```python
from build123d import *

# Parameters (mm, degrees)
SHAFT_SECTION_A_PROFILE_10_R = 5
SHAFT_SECTION_A_10X64_DEPTH  = 64
COLLAR_PROFILE_24_R          = 12
COLLAR_24X2_DEPTH            = 2
SHAFT_START                  = 80
SHAFT_SECTION_B_PROFILE_10_R = 5
SHAFT_SECTION_B_10X80_DEPTH  = 80
HEAD_PROFILE_18_R            = 9
HEAD_18X4_DEPTH              = 4


with BuildPart() as part:
    # Shaft Section A Profile Ø10 → Shaft Section A Ø10x64 (new body)
    with BuildSketch(Plane(origin=(0, 0, 0), x_dir=(0, 0, -1), z_dir=(1, 0, 0))):
        Circle(SHAFT_SECTION_A_PROFILE_10_R)
    extrude(amount=SHAFT_SECTION_A_10X64_DEPTH)

    # Collar Profile Ø24 → Collar Ø24x2 (add)
    with BuildSketch(Plane.ZY):
        Circle(COLLAR_PROFILE_24_R)
    extrude(amount=COLLAR_24X2_DEPTH)

    # Shaft Section B Profile Ø10 → Shaft Section B Ø10x80 (add)
    with BuildSketch(Plane.ZY.offset(2).offset(SHAFT_START)):
        with Locations(Location((0, 0, 0), (0, 0, 180))):
            Circle(SHAFT_SECTION_B_PROFILE_10_R)
    extrude(amount=-SHAFT_SECTION_B_10X80_DEPTH)

    # Head Profile Ø18 → Head Ø18x4 (add)
    with BuildSketch(Plane.ZY.offset(82)):
        Circle(HEAD_PROFILE_18_R)
    extrude(amount=HEAD_18X4_DEPTH)


solid = part.part
```
Geometry check sheet. Reference: the model listing, model coordinates, mm. A direction names the side the tool comes from. Round coordinates to 2 decimals unless told otherwise and drop trailing zeros. Order: outer loops, then holes, each group sorted by start corner. A loop starts at its lowest first (then second) coordinate and runs counter-clockwise, first axis right, second up. Notation, with made-up numbers: (37.5, 31) - (83.5, 31) arc R27 cw to (83.5, 52) - close; hole circle Ø8 at (45.25, 23.25). An arc over 180 degrees is marked (long way). Use a Markdown table: item, result. Add a question column.
(1) Sectioned sample at A-A, the plane y = 7.5. Enter the section's corners in (x, z), and give its area (3 significant figures).
(2) Tool access check on faces 1 (the flat face through (64, 0, 0)), 2 (the flat face through (-86, 0, 0)), 3 (the cylindrical face through (-83.972, 8.923, -1.172)), 4 (the flat face through (-2, 0.2, 5.2)), 5 (the flat face through (0, 0.2, 5.2)). Record the directions out of +Z, -Z, +X, -X, +Y, -Y that give a thin tool (end or side, any length) a straight path to the whole face; none if there is none.
(3) Depth check by flat-ended pin: pin 1 (2 mm diameter, centred on x = 42.5, z = -5.5, fed in from -Y); pin 2 (4 mm diameter, centred on x = 39, y = 8.5, fed in from -Z); pin 3 (4 mm diameter, centred on x = 17.5, z = 6.5, fed in from +Y); pin 4 (5 mm diameter, centred on x = 48, y = -5, fed in from +Z). Enter the tip coordinate at first touch or a pass-through.
(4) Sectioned sample at C-C, the plane z = 6.5. Enter the section's corners in (x, y), and give its area (3 significant figures).
(5) Sectioned sample at B-B, the plane z = 0. Enter the section's corners in (x, y).
(6) Material ranges on line 1 along X through (y, z) = (0.5, 8.25); line 2 along X through (y, z) = (-10.5, 3); line 3 along Z through (x, y) = (49, 0.5), recorded low to high. Write a range as [from, to].
Answers below:
| question | item | result |
|---|---|---|
| 1 | outline | (-86, -4.97) - (-82, -4.97) - (-82, 4.97) - (-86, 4.97) - close; (-2, -9.37) - (0, -9.37) - (0, 9.37) - (-2, 9.37) - close |
| 1 | area | 77.3 mm² |
| 2 | face 1 | +Z, -Z, +X, +Y, -Y |
| 2 | face 2 | +Z, -Z, -X, +Y, -Y |
| 2 | face 3 | -X |
| 2 | face 4 | none |
| 2 | face 5 | +X |
| 3 | pin 1 | y = -2.18 |
| 3 | pin 2 | through |
| 3 | pin 3 | y = 2.18 |
| 3 | pin 4 | z = 4.33 |
| 4 | outline | (-86, -6.22) - (-82, -6.22) - (-82, 6.22) - (-86, 6.22) - close; (-2, -10.09) - (0, -10.09) - (0, 10.09) - (-2, 10.09) - close |
| 4 | area | 90.1 mm² |
| 5 | outline | (-86, -9) - (-82, -9) - (-82, -5) - (-2, -5) - (-2, -12) - (0, -12) - (0, -5) - (64, -5) - (64, 5) - (0, 5) - (0, 12) - (-2, 12) - (-2, 5) - (-82, 5) - (-82, 9) - (-86, 9) - close |
| 6 | line 1 | [-86, -82], [-2, 0] |
| 6 | line 2 | [-2, 0] |
| 6 | line 3 | [-4.97, 4.97] |
